from build123d import *

# Parameters (mm, degrees)
SKETCH1_R           = 5
BOSS_EXTRUDE1_DEPTH = 1.5
SKETCH2_R           = 3
BOSS_EXTRUDE2_DEPTH = 8
BOSS_EXTRUDE3_START = 3
SKETCH3_R           = 3
BOSS_EXTRUDE3_DEPTH = 3
CHAMFER1_SIZE       = 0.2


with BuildPart() as part:
    # Sketch1 → Boss-Extrude1 (new body)
    with BuildSketch(Plane(origin=(0, 0, 0), x_dir=(1, 0, 0), z_dir=(0, 1, 0))):
        with Locations(Location((0, 0, 0), (0, 0, 270))):
            Circle(SKETCH1_R)
    extrude(amount=BOSS_EXTRUDE1_DEPTH)

    # Sketch2 → Boss-Extrude2 (add)
    with BuildSketch(Plane(origin=(0, 1.5, 0), x_dir=(1, 0, 0), z_dir=(0, 1, 0))):
        with Locations(Location((0, 0, 0), (0, 0, 270))):
            Circle(SKETCH2_R)
    extrude(amount=BOSS_EXTRUDE2_DEPTH)

    # Sketch3 → Boss-Extrude3 (add)
    with BuildSketch(Plane.XZ.offset(BOSS_EXTRUDE3_START)):
        with Locations(Location((0, 0, 0), (0, 0, 90))):
            Circle(SKETCH3_R)
    extrude(amount=-BOSS_EXTRUDE3_DEPTH)

    # Chamfer1
    chamfer1_edges = [part.edges().sort_by_distance(p)[0] for p in [
        (0, -3, -3),
        (0, 0, -5),
        (0, 1.5, -5),
        (0, 9.5, -3),
    ]]
    chamfer(chamfer1_edges, length=CHAMFER1_SIZE)


solid = part.part
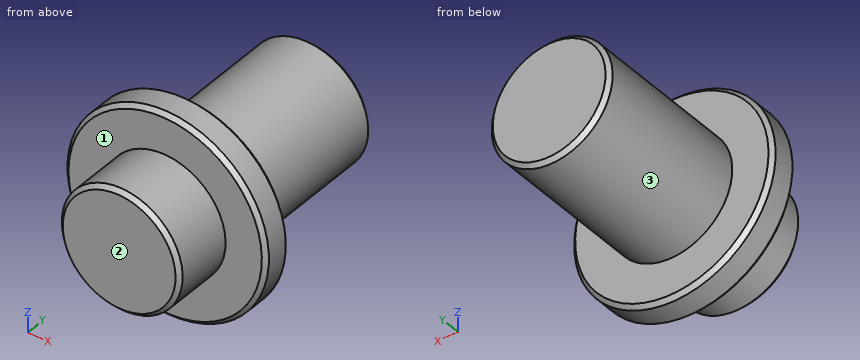
Verification items for the finished model (mm, model axes). Face numbers are marked on the shaded views. A direction names the side the tool comes from. Give positions to 0.01 mm unless a question says otherwise; leave off trailing zeros. Order: outer loops, then holes, each group sorted by start corner. A loop starts at its lowest first (then second) coordinate and runs counter-clockwise, first axis right, second up. Notation, with made-up numbers: M 36,-5 L 65,-5 A28 cw 65,33 Z; hole C 79.25,46 d3. An arc over 180 degrees is marked long. Use one line per item in the form item = value. Start each with the question number.
Q1. Section check C-C (y = 8.5). Enter the section's corners in (x, z).
Q2. Scan lines: line 1 along Y through (x, z) = (-4, -0.5); line 2 along X through (y, z) = (8.5, 0); line 3 along X through (y, z) = (1, -4.25). Record each from-to range of solid material in increasing order. Write a range as [from, to].
Q3. Section check B-B (x = 0). Enter the section's corners in (y, z), then the cut area to 3 significant figures.
Q4. Section check A-A (z = 0). Enter the section's corners in (x, y), then the cut area to 3 significant figures.
Q5. Go/stop test with flat-tipped pins: pin 1 Ø6 at (x, y) = (1.5, 6.5) entering from +Z; pin 2 Ø1 at (x, y) = (-2.5, 4.5) entering from +Z; pin 3 Ø3 at (x, y) = (3.5, 5) entering from -Z; pin 4 Ø5 at (x, z) = (-2.5, -2) entering from -Y. Record where each tip stops, or that it passes through.
Q6. Access from +Z, -Z, +X, -X, +Y, -Y to the whole of each face (thin tool, end or side, straight path). Record for the marked faces 1, 2 and 3.
Evaluation:
q1.outline = C 0,0 d6
q2.line_1 = [0, 1.5]
q2.line_2 = [-3, 3]
q2.line_3 = [-2.63, 2.63]
q3.outline = M -3,-2.8 L -2.8,-3 L 0,-3 L 0,-4.8 L 0.2,-5 L 1.3,-5 L 1.5,-4.8 L 1.5,-3 L 9.3,-3 L 9.5,-2.8 L 9.5,2.8 L 9.3,3 L 1.5,3 L 1.5,4.8 L 1.3,5 L 0.2,5 L 0,4.8 L 0,3 L -2.8,3 L -3,2.8 Z
q3.area = 80.8 mm2
q4.outline = M -5,0.2 L -4.8,0 L -3,0 L -3,-2.8 L -2.8,-3 L 2.8,-3 L 3,-2.8 L 3,0 L 4.8,0 L 5,0.2 L 5,1.3 L 4.8,1.5 L 3,1.5 L 3,9.3 L 2.8,9.5 L -2.8,9.5 L -3,9.3 L -3,1.5 L -4.8,1.5 L -5,1.3 Z
q4.area = 80.8 mm2
q5.pin_1 = 3
q5.pin_2 = 2.24
q5.pin_3 = -2.24
q5.pin_4 = -3
q6.face_1 = -Y
q6.face_2 = +Z, -Z, +X, -X, -Y
q6.face_3 = +Y
